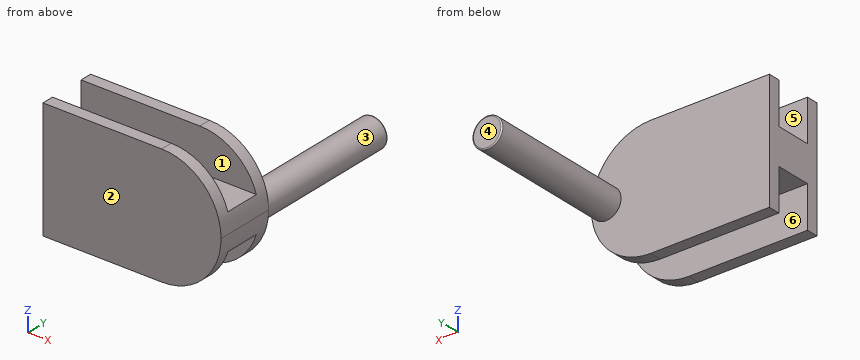
```python
from build123d import *

# Parameters (mm, degrees)
SKETCH1_W           = 30
SKETCH1_H           = 20
BOSS_EXTRUDE1_DEPTH = 10
SKETCH2_W           = 7
SKETCH2_H           = 6
CUT_EXTRUDE1_DEPTH  = 38.416573868
CUT_EXTRUDE2_DEPTH  = 38.416573868
SKETCH4_R           = 2.5
BOSS_EXTRUDE2_DEPTH = 25
FILLET1_R           = 0.2


with BuildPart() as part:
    # Sketch1 → Boss-Extrude1 (new body)
    with BuildSketch(Plane(origin=(0, 0, 0), x_dir=(1, 0, 0), z_dir=(0, 1, 0))):
        with Locations((15, 10)):
            Rectangle(SKETCH1_W, SKETCH1_H)
    extrude(amount=BOSS_EXTRUDE1_DEPTH)

    # Sketch2 → Cut-Extrude1 (cut, through all)
    with BuildSketch(Plane.ZY):
        with Locations((-16.5, 5)):
            Rectangle(SKETCH2_W, SKETCH2_H)
        with Locations((-3.5, 5)):
            Rectangle(SKETCH2_W, SKETCH2_H)
    extrude(amount=-CUT_EXTRUDE1_DEPTH, mode=Mode.SUBTRACT)

    # Sketch3 → Cut-Extrude2 (cut, through all)
    with BuildSketch(Plane(origin=(0, 10, 0), x_dir=(1, 0, 0), z_dir=(0, 1, 0))):
        with BuildLine():
            Line((30, 0), (30, 10))
            ThreePointArc((30, 10), (27.071067812, 2.928932188), (20, 0))
            Line((20, 0), (30, 0))
        make_face()
        with BuildLine():
            Line((30, 10), (30, 20))
            Line((30, 20), (20, 20))
            ThreePointArc((20, 20), (27.071067812, 17.071067812), (30, 10))
        make_face()
    extrude(amount=-CUT_EXTRUDE2_DEPTH, mode=Mode.SUBTRACT)

    # Sketch4 → Boss-Extrude2 (add)
    with BuildSketch(Plane(origin=(0, 10, 0), x_dir=(1, 0, 0), z_dir=(0, 1, 0))):
        with Locations(Location((27.5, 10, 0), (0, 0, 359.999408267))):
            Circle(SKETCH4_R)
    extrude(amount=BOSS_EXTRUDE2_DEPTH)

    # Fillet1
    fillet1_edges = [part.edges().sort_by_distance(p)[0] for p in [
        (25, 35, -10.000025819),
    ]]
    fillet(fillet1_edges, radius=FILLET1_R)


solid = part.part
```
The model under review builds one solid part; all positions refer to its coordinate system, in mm. Face numbers are marked on the shaded views. A direction names the side the tool comes from. Round coordinates to 2 decimals unless told otherwise and drop trailing zeros. Write each loop counter-clockwise with the first axis right and the second up, starting at its lowest first coordinate (ties: lowest second). Pieces come first, ordered by that corner, then holes. Notation, with made-up numbers: M -16,-8 L 33,-8 A7 ccw 33,-1 Z; hole C 88,-29.5 d8. An arc over 180 degrees is marked long. Use CSV: the item, a comma, the result in double quotes. Start each with the question number.
(1) We need section D-D, the plane z = -3.75. State the section outline as (x, y) points.
(2) We need section A-A, the plane z = -14.25. State the section outline as (x, y) points.
(3) Clearance check with flat-ended pins moving along their axes: P1, Ø5, axis at x = 12.5, y = 5, coming from the +Z side; P2, Ø12, axis at x = 26.5, y = 10.5, coming from the -Z side; P3, Ø8, axis at x = 24.5, y = 26, coming from the +Z side. State where each tip first meets the part, or that it passes through.
(4) For line 1 along Y through (x, z) = (3, -16.75); line 2 along X through (y, z) = (13, -10); line 3 along Y through (x, z) = (21, -7.75), list the stretches that pass through material, from the lowest coordinate up.
(5) Tool access review of the marked faces 4, 5 and 6: name each direction out of +Z, -Z, +X, -X, +Y, -Y from which nothing blocks a thin tool from reaching the whole face with its end or side.
(6) We need section B-B, the plane x = 23. State the section outline as (y, z) points.
(7) We need section C-C, the plane y = 9. State the section outline as (x, z) points, then the cut area to 3 significant figures.
(8) The part is to be moulded in two halves that separate along Y. For the marked faces 1, 2 and 3, say which applies: +Y half, -Y half, draft (parallel to the pull), parting line (faces both ways), or undercut.
Findings:
1,outline,"M 0,0 L 27.81,0 L 27.81,2 L 0,2 Z; M 0,8 L 27.81,8 L 27.81,10 L 0,10 Z"
2,outline,"M 0,0 L 29.05,0 L 29.05,2 L 0,2 Z; M 0,8 L 29.05,8 L 29.05,10 L 0,10 Z"
3,P1,"z = -7"
3,P2,"z = -19.99"
3,P3,"z = -7.5"
4,line 1,"0 to 2, 8 to 10"
4,line 2,"25 to 30"
4,line 3,"0 to 10"
5,face 4,"+Z, -Z, +X, -X, +Y"
5,face 5,"+Z, +X, -X"
5,face 6,"-Z, +X, -X"
6,outline,"M 0,-19.54 L 2,-19.54 L 2,-13 L 8,-13 L 8,-19.54 L 10,-19.54 L 10,-0.46 L 8,-0.46 L 8,-7 L 2,-7 L 2,-0.46 L 0,-0.46 Z"
7,outline,"M 0,-20 L 20,-20 A10 ccw 20,0 L 0,0 Z"
7,area,"557 mm^2"
8,face 1,"undercut"
8,face 2,"-Y half"
8,face 3,"draft"
